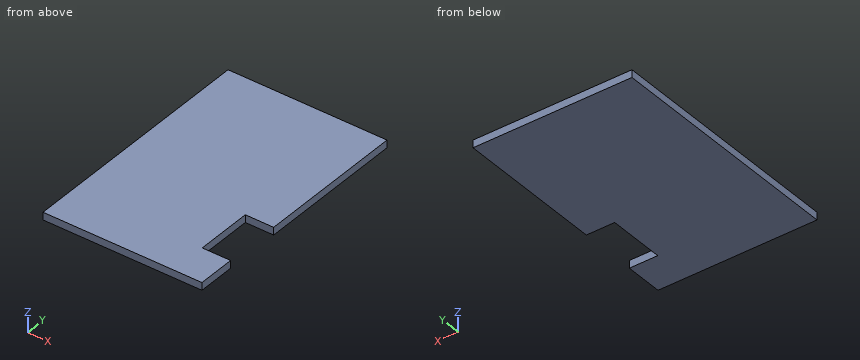
from build123d import *

# Parameters (mm, degrees)
BOSS_EXTRUDE1_DEPTH = 40


with BuildPart() as part:
    # Sketch1 → Boss-Extrude1 (new body)
    with BuildSketch(Plane.XY):
        Polygon((0, 0), (840, 0), (840, 200), (690, 200), (690, 500), (840, 500), (840, 1290), (0, 1290), align=None)
    extrude(amount=BOSS_EXTRUDE1_DEPTH)


solid = part.part
Part model, mm, in its own coordinate system. Give positions to 0.01 mm unless a question says otherwise; leave off trailing zeros. Write each loop counter-clockwise with the first axis right and the second up, starting at its lowest first coordinate (ties: lowest second). Pieces come first, ordered by that corner, then holes.
1) Probe L1, parallel to Y at x = 766, z = 19; L2, parallel to X at y = 451, z = 12. List the from-to ranges inside material, lowest first.
Resolved:
L1: y = 0 to 200, 500 to 1290
L2: x = 0 to 690
2) Pin check, flat tip, straight feed: pin 1 (12 mm diameter, centred on y = 314.5, z = 25.5, fed in from +X). Stop position of the tip, or through.
Resolved:
pin 1: stops at x = 690
3) Cut at B-B on y = 347.5. Write the cut outline in (x, z).
Resolved:
outline: (0, 0) - (690, 0) - (690, 40) - (0, 40) - close
4) Cut at A-A on z = 30. Write the cut outline in (x, y), then the cut area to 3 significant figures.
Resolved:
outline: (0, 0) - (840, 0) - (840, 200) - (690, 200) - (690, 500) - (840, 500) - (840, 1290) - (0, 1290) - close
area: 1,040,000 mm2
